Geometry check sheet. Reference: drawing and pictorial views, mm from the part's lowest x, y, z. Give positions to 0.01 mm unless a question says otherwise; leave off trailing zeros. Write each loop counter-clockwise with the first axis right and the second up, starting at its lowest first coordinate (ties: lowest second). Pieces come first, ordered by that corner, then holes.
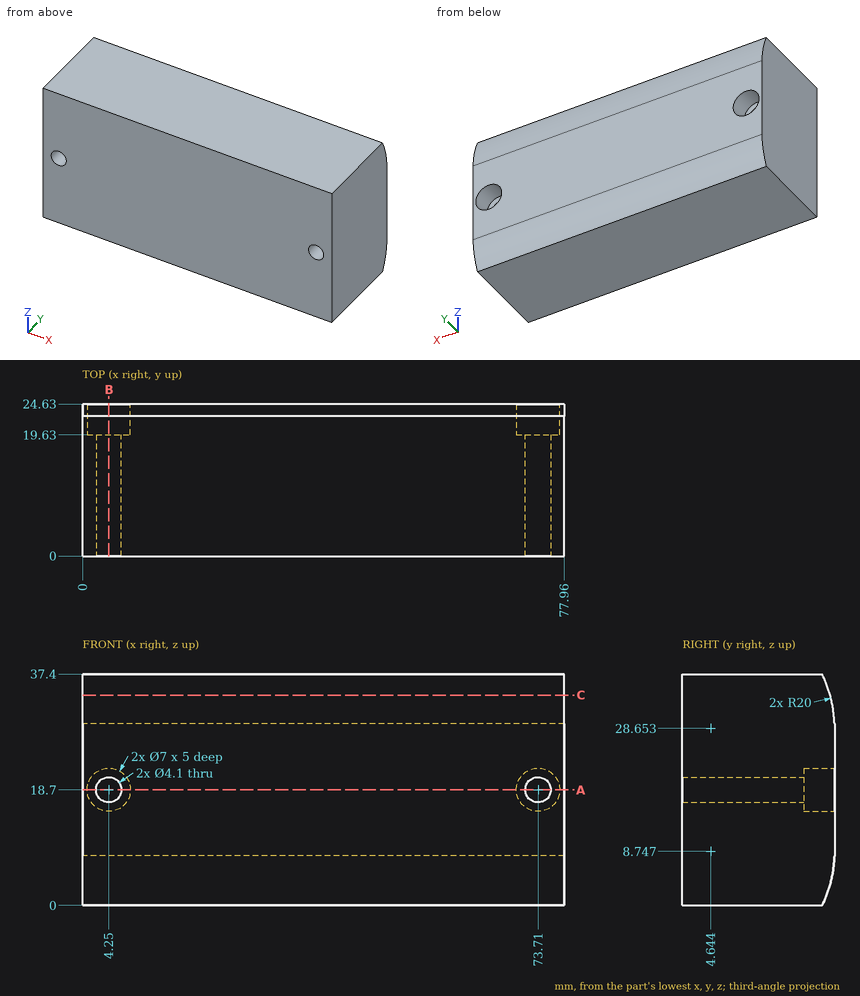
Item 1: Depth check by flat-ended pin: pin 1 (2 mm diameter, centred on x = 72.5, z = 18.5, fed in from +Y); pin 2 (12 mm diameter, centred on x = 8.5, z = 30, fed in from -Y). Enter the tip coordinate at first touch or a pass-through.
Answer key:
pin 1: stops at y = 19.63
pin 2: stops at y = 0
Item 2: Sectioned sample at B-B on x = 4.25. Record the cut outline in (y, z).
Answer key:
outline: (0, 0) - (22.63, 0) arc R20 ccw to (24.63, 8) - (24.63, 15.2) - (19.63, 15.2) - (19.63, 16.65) - (0, 16.65) - close; (0, 20.75) - (19.63, 20.75) - (19.63, 22.2) - (24.63, 22.2) - (24.63, 29.4) arc R20 ccw to (22.63, 37.4) - (0, 37.4) - close
Item 3: Scan lines: line 1 along Z through (x, y) = (4.25, 20.7); line 2 along Z through (x, y) = (4.25, 12.75); line 3 along X through (y, z) = (1.5, 17) (1 decimal). Record each from-to range of solid material in increasing order.
Answer key:
line 1: z = 0 to 15.2, 22.2 to 37.4
line 2: z = 0 to 16.65, 20.75 to 37.4
line 3: x = 0 to 3.1, 5.4 to 72.6, 74.9 to 78
Item 4: Sectioned sample at A-A on z = 18.7. Record the cut outline in (x, y), then the cut area to 3 significant figures.
Answer key:
outline: (0, 0) - (2.2, 0) - (2.2, 19.63) - (0.75, 19.63) - (0.75, 24.63) - (0, 24.63) - close; (6.3, 0) - (71.66, 0) - (71.66, 19.63) - (70.21, 19.63) - (70.21, 24.63) - (7.75, 24.63) - (7.75, 19.63) - (6.3, 19.63) - close; (75.76, 0) - (77.96, 0) - (77.96, 24.63) - (77.21, 24.63) - (77.21, 19.63) - (75.76, 19.63) - close
area: 1,690 mm2
Item 5: Sectioned sample at C-C on z = 34. Record the cut outline in (x, y), then the cut area to 3 significant figures.
Answer key:
outline: (0, 0) - (77.96, 0) - (77.96, 23.92) - (0, 23.92) - close
area: 1,860 mm2
